The model under review builds one solid part; all positions refer to its coordinate system, in mm. Coordinates: 2 decimals unless noted, no trailing zeros. Order: outer loops, then holes, each group sorted by start corner. A loop starts at its lowest first (then second) coordinate and runs counter-clockwise, first axis right, second up. Notation, with made-up numbers: (-20, 16.25) -> (-14, 16.25) arc R14 cw to (-14, 37.25) -> close; hole circle Ø4 at (37.25, -9). An arc over 180 degrees is marked (long way). Use one line per item in the form item = value.
from build123d import *

# Parameters (mm, degrees)
SKETCH1_W             = 150
SKETCH1_H             = 100
BOSS_EXTRUDE1_DEPTH   = 15
M8_TAPPED_HOLE1_D     = 6.8
M8_TAPPED_HOLE1_DEPTH = 19.75
M8_TAPPED_HOLE1_TIP   = 2.042926105


with BuildPart() as part:
    # Sketch1 → Boss-Extrude1 (new body)
    with BuildSketch(Plane.XY):
        Rectangle(SKETCH1_W, SKETCH1_H)
    extrude(amount=BOSS_EXTRUDE1_DEPTH)

    # M8 Tapped Hole1
    with Locations(Plane.XY.offset(15)):
        with Locations((4.354174377, 16.25), (60.645825623, 16.25), (32.5, -32.5)):
            Hole(M8_TAPPED_HOLE1_D / 2, depth=M8_TAPPED_HOLE1_DEPTH)
            with Locations((0, 0, -(M8_TAPPED_HOLE1_DEPTH + M8_TAPPED_HOLE1_TIP / 2))):  # 118° drill point
                Cone(0, M8_TAPPED_HOLE1_D / 2, M8_TAPPED_HOLE1_TIP, mode=Mode.SUBTRACT)


solid = part.part
Item 1: Clearance check with a flat-ended pin moving along its axis: pin 1 (5 mm diameter, centred on x = -10, y = 19, fed in from -Z). State where the tip first meets the part, or that it passes through.
Results found:
pin_1 = 0
Item 2: We need section A-A (y = 16.25). Write out the cut boundary in (x, z), plus the area to 3 significant figures.
Results found:
outline = (-75, 0) -> (0.95, 0) -> (0.95, 15) -> (-75, 15) -> close; (7.75, 0) -> (57.25, 0) -> (57.25, 15) -> (7.75, 15) -> close; (64.05, 0) -> (75, 0) -> (75, 15) -> (64.05, 15) -> close
area = 2,050 mm²
Item 3: We need section B-B (x = 32.5). Write out the cut boundary in (y, z), plus the area to 3 significant figures.
Results found:
outline = (-50, 0) -> (-35.9, 0) -> (-35.9, 15) -> (-50, 15) -> close; (-29.1, 0) -> (50, 0) -> (50, 15) -> (-29.1, 15) -> close
area = 1,400 mm²
Item 4: To check wall thickness, follow L1, parallel to X at y = -33, z = 11; L2, parallel to Y at x = 32.5, z = 11.75; L3, parallel to Y at x = 35, z = 11.25. State the ranges of each line that lie inside material, in increasing order. Write a range as from..to.
Results found:
L1 = -75..29.14, 35.86..75
L2 = -50..-35.9, -29.1..50
L3 = -50..-34.8, -30.2..50
Item 5: We need section C-C (x = 5). Write out the cut boundary in (y, z), plus the area to 3 significant figures.
Results found:
outline = (-50, 0) -> (12.91, 0) -> (12.91, 15) -> (-50, 15) -> close; (19.59, 0) -> (50, 0) -> (50, 15) -> (19.59, 15) -> close
area = 1,400 mm²
